Input: dimensioned drawing with shaded views. Units: mm. Origin: part minimum x, y, z. A direction names the side the tool comes from. Round coordinates to 2 decimals unless told otherwise and drop trailing zeros. Loops run counter-clockwise (first coordinate to the right, second up) from the corner with the lowest first, then second, coordinate; pieces in that order, holes last. Notation, with made-up numbers: M 73,-14 L 100,-14 A35 cw 100,20 Z; hole C 61.25,-9.5 d9. An arc over 180 degrees is marked long. Use one line per item in the form item = value. Start each with the question number.
Q1. Section query D-D, the plane y = 76. Output: boundary loops of the cut face in (x, z).
Q2. Ray query, line 1 along X through (y, z) = (19, 15); line 2 along X through (y, z) = (9.5, 12); line 3 along Z through (x, y) = (63, 56). Return the intervals inside material, ascending.
Q3. First-contact query: P1, Ø12, axis at x = 133.5, y = 124, coming from the -Z side; P2, Ø2, axis at x = 63.5, y = 62, coming from the +Z side; P3, Ø9, axis at y = 62, z = 8.5, coming from the -X side. Flat tips, straight axial feed; report the tip coordinate or a pass-through.
Q4. Section query A-A, the plane x = 15. Output: boundary loops of the cut face in (y, z), and give its area (3 significant figures).
Q5. Access query for the marked faces 1, 2 and 3. Directions: +Z, -Z, +X, -X, +Y, -Y. A direction counts if a zero-diameter tool reaches every point of the face in a straight line with its end or side. Return the directions, or none.
Q6. Section query B-B, the plane z = 15. Output: boundary loops of the cut face in (x, y), and give its area (3 significant figures).
Q7. Section query C-C, the plane y = 9. Output: boundary loops of the cut face in (x, z).
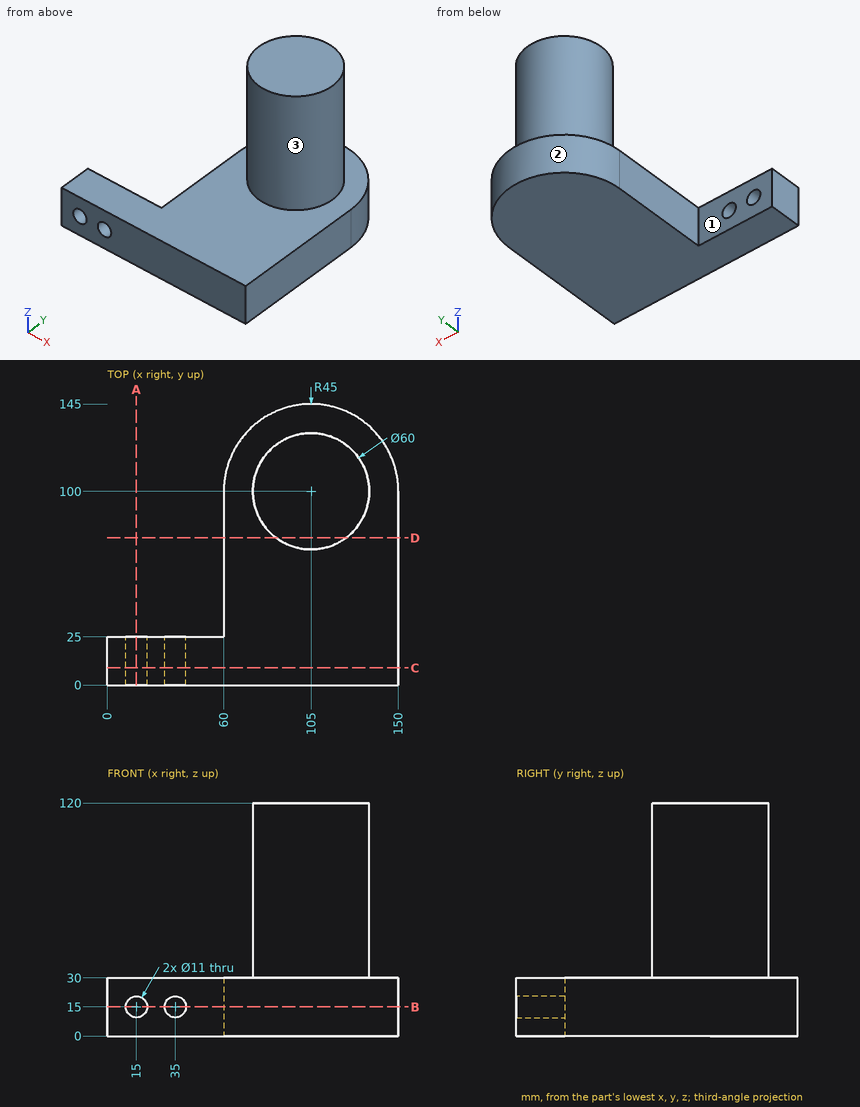
Results found:
q1.outline = M 60,0 L 150,0 L 150,30 L 123,30 L 123,120 L 87,120 L 87,30 L 60,30 Z
q2.line_1 = 0 to 9.5, 20.5 to 29.5, 40.5 to 150
q2.line_2 = 0 to 10.39, 19.61 to 30.39, 39.61 to 150
q2.line_3 = 0 to 30
q3.P1 = 0
q3.P2 = 30
q3.P3 = 60
q4.outline = M 0,0 L 25,0 L 25,9.5 L 0,9.5 Z; M 0,20.5 L 25,20.5 L 25,30 L 0,30 Z
q4.area = 475 mm²
q5.face_1 = +Z, -Z, -X, +Y
q5.face_2 = +Z, -Z, +Y
q5.face_3 = +Z
q6.outline = M 0,0 L 9.5,0 L 9.5,25 L 0,25 Z; M 20.5,0 L 29.5,0 L 29.5,25 L 20.5,25 Z; M 40.5,0 L 150,0 L 150,100 A45 ccw 60,100 L 60,25 L 40.5,25 Z
q6.area = 13,100 mm²
q7.outline = M 0,0 L 150,0 L 150,30 L 0,30 Z; hole C 15,15 d11; hole C 35,15 d11
